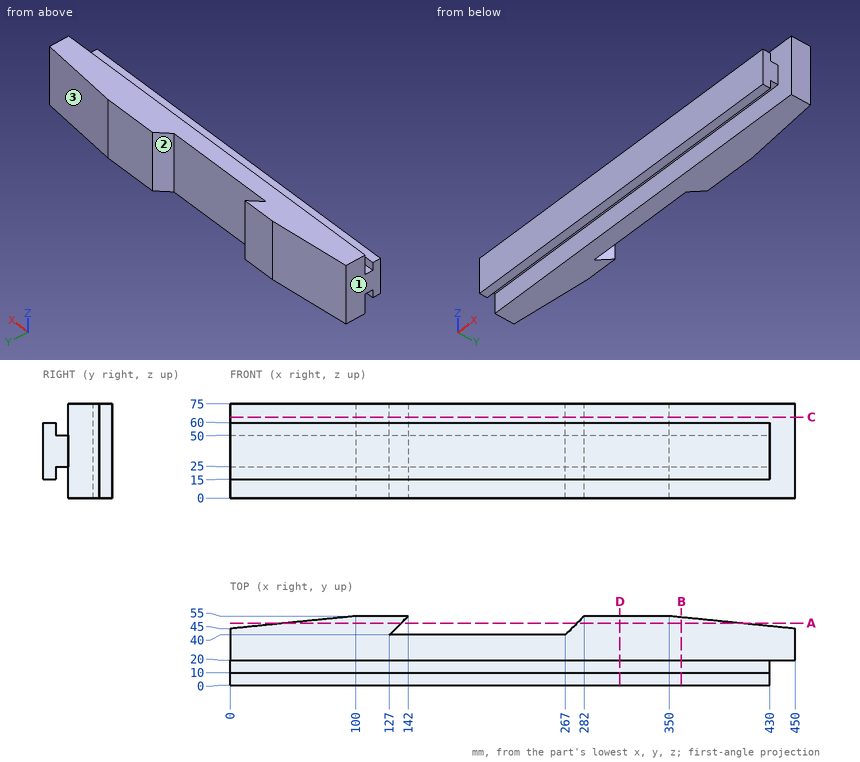
Input: dimensioned drawing with shaded views. Units: mm. Origin: part minimum x, y, z. Give positions to 0.01 mm unless a question says otherwise; leave off trailing zeros. Write each loop counter-clockwise with the first axis right and the second up, starting at its lowest first coordinate (ties: lowest second). Pieces come first, ordered by that corner, then holes. Notation, with made-up numbers: (61, 8) -> (76, 8) arc R15 ccw to (76, 34) -> close; hole circle Ø1 at (-37.5, -25). An arc over 180 degrees is marked (long way). Answer as a JSON object with one key per item and string values.
1. Cut plane A-A on y = 49.5. Output: boundary loops of the cut face in (x, z).
Ans:
{"outline": "(45, 0) -> (136.5, 0) -> (136.5, 75) -> (45, 75) -> close; (276.5, 0) -> (405, 0) -> (405, 75) -> (276.5, 75) -> close"}
2. Cut plane B-B on x = 359.5. Output: boundary loops of the cut face in (y, z).
Ans:
{"outline": "(0, 15) -> (10, 15) -> (10, 25) -> (20, 25) -> (20, 0) -> (54.05, 0) -> (54.05, 75) -> (20, 75) -> (20, 50) -> (10, 50) -> (10, 60) -> (0, 60) -> close"}
3. Contact query for flat-ended pins moving along their axis: pin 1 (8 mm diameter, centred on x = 191.5, y = 13.5, fed in from +Z); pin 2 (5 mm diameter, centred on y = 34.5, z = 30.5, fed in from -X); pin 3 (1 mm diameter, centred on x = 405, z = 25, fed in from +Y); pin 4 (3 mm diameter, centred on x = 202.5, y = 5.5, fed in from -Z). Output: stop coordinate, or through.
Ans:
{"pin 1": "stops at z = 60", "pin 2": "stops at x = 0", "pin 3": "stops at y = 49.55", "pin 4": "stops at z = 15"}
4. Mould query, pull axis X, two halves, no side actions, for the marked faces 1, 2 and 3. Classes: pulls with the +X half, pulls with the -X half, needs draft (parallel to the pull), parting line crosses it, or undercut.
Ans:
{"face 1": "pulls with the -X half", "face 2": "undercut", "face 3": "pulls with the +X half"}
5. Ray query, probe 1 along Z at (x, y) = (358, 4); probe 2 along X at (y, z) = (19.5, 31); probe 3 along Y at (x, z) = (195.5, 35). Return the intervals inside material, ascending. Write a range as from..to.
Ans:
{"probe 1": "z = 15..60", "probe 2": "x = 0..430", "probe 3": "y = 0..40"}
6. Cut plane C-C on z = 64.5. Output: boundary loops of the cut face in (x, y).
Ans:
{"outline": "(0, 20) -> (450, 20) -> (450, 45) -> (350, 55) -> (282, 55) -> (267, 40) -> (127, 40) -> (142, 55) -> (100, 55) -> (0, 45) -> close"}
7. Cut plane D-D on x = 310.5. Output: boundary loops of the cut face in (y, z), and give its area (4 significant figures).
Ans:
{"outline": "(0, 15) -> (10, 15) -> (10, 25) -> (20, 25) -> (20, 0) -> (55, 0) -> (55, 75) -> (20, 75) -> (20, 50) -> (10, 50) -> (10, 60) -> (0, 60) -> close", "area": "3,325 mm^2"}
